Build history of the part. All positions in model axes, mm. Face numbers are marked on the shaded views. A direction names the side the tool comes from. Coordinates: 2 decimals unless noted, no trailing zeros. Order: outer loops, then holes, each group sorted by start corner. A loop starts at its lowest first (then second) coordinate and runs counter-clockwise, first axis right, second up. Notation, with made-up numbers: (10, 72.25) -> (45, 72.25) arc R7 cw to (45, 78.25) -> close; hole circle Ø3 at (-36.5, 22). An arc over 180 degrees is marked (long way). Write each question's results on one line, items separated by ' | '.
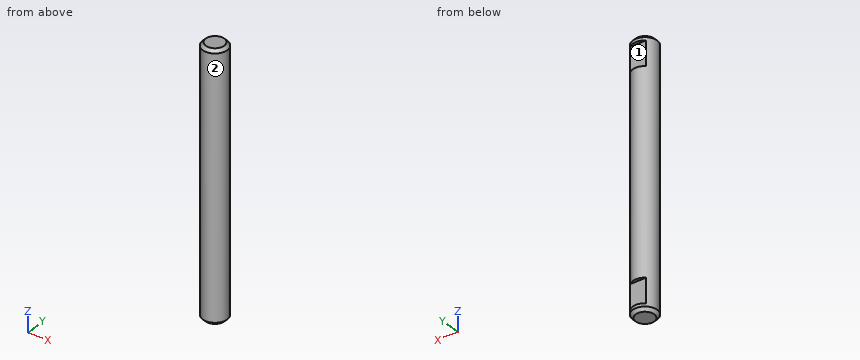
from build123d import *

# Parameters (mm, degrees)
SKETCH1_R           = 2
BOSS_EXTRUDE1_DEPTH = 21.5
SKETCH2_W           = 15.41853157
SKETCH2_H           = 4
SKETCH2_W_2         = 11.817796653
CUT_EXTRUDE1_DEPTH  = 0.5
CHAMFER1_SIZE       = 0.5


with BuildPart() as part:
    # Sketch1 → Boss-Extrude1 (new, symmetric)
    with BuildSketch(Plane.XY):
        Circle(SKETCH1_R)
    extrude(amount=BOSS_EXTRUDE1_DEPTH, both=True)

    # Sketch2 → Cut-Extrude1 (cut)
    with BuildSketch(Plane(origin=(0, 2, 0), x_dir=(-1, 0, 0), z_dir=(0, 1, 0))):
        with Locations((0, 18.5)):
            Rectangle(SKETCH2_W, SKETCH2_H)
        with Locations((0.877102096, -18.5)):
            Rectangle(SKETCH2_W_2, SKETCH2_H)
    extrude(amount=-CUT_EXTRUDE1_DEPTH, mode=Mode.SUBTRACT)

    # Chamfer1
    chamfer1_edges = [part.edges().sort_by_distance(p)[0] for p in [
        (-2, 0, -21.5),
        (-2, 0, 21.5),
    ]]
    chamfer(chamfer1_edges, length=CHAMFER1_SIZE)


solid = part.part
Item 1: Tool access for the marked faces 1 and 2: list every direction of +Z, -Z, +X, -X, +Y, -Y with a clear straight run to the whole face (end or side of a thin tool).
Answer:
face 1: +X, -X, +Y | face 2: +Z, -Z
Item 2: Slice it at C-C, the plane z = 3. List the corners of the cut face in (x, y), and give its area (3 significant figures).
Answer:
outline: circle Ø4 at (0, 0) | area: 12.6 mm^2
Item 3: Slice it at B-B, the plane z = -17. List the corners of the cut face in (x, y), and give its area (3 significant figures).
Answer:
outline: (-1.32, 1.5) arc R2 ccw (long way) to (1.32, 1.5) -> close | area: 11.7 mm^2
Item 4: Pin check, flat tips, straight feed: pin 1 (0.6 mm diameter, centred on x = -0.5, y = 2, fed in from +Z); pin 2 (2 mm diameter, centred on x = 0.5, z = 18, fed in from +Y). Stop position of each tip, or through.
Answer:
pin 1: stops at z = 21.24 | pin 2: stops at y = 1.5
Item 5: Drill centre lines: line 1 (Y direction, x = 0.15, z = -20); line 2 (X direction, y = -0.3, z = 9); line 3 (Y direction, x = 1.2, z = 17). Where is each one in solid material? Low to high. Write a range as from..to.
Answer:
line 1: y = -1.99..1.5 | line 2: x = -1.98..1.98 | line 3: y = -1.6..1.5
Item 6: Slice it at A-A, the plane x = 0. List the corners of the cut face in (y, z).
Answer:
outline: (-2, -21) -> (-1.5, -21.5) -> (1.5, -21.5) -> (2, -21) -> (2, -20.5) -> (1.5, -20.5) -> (1.5, -16.5) -> (2, -16.5) -> (2, 16.5) -> (1.5, 16.5) -> (1.5, 20.5) -> (2, 20.5) -> (2, 21) -> (1.5, 21.5) -> (-1.5, 21.5) -> (-2, 21) -> close
